Here's how the part is built. I have some questions about the finished solid (model axes, mm). A direction names the side the tool comes from. Round coordinates to 2 decimals unless told otherwise and drop trailing zeros. Write each loop counter-clockwise with the first axis right and the second up, starting at its lowest first coordinate (ties: lowest second). Pieces come first, ordered by that corner, then holes. Notation, with made-up numbers: (-26.75, 70) - (19.25, 70) arc R9 cw to (19.25, 86) - close; hole circle Ø7 at (64, 83). An arc over 180 degrees is marked (long way). One line per question, with ' | ' between items. Start each with the question number.
(1) For faces 4 (the flat face through (-12.5, 0, 5)), 5 (the flat face through (0, 7, 0.5)), 6 (the cylindrical face through (9.6, -4.3, 7.5)), which set-ups out of +Z, -Z, +X, -X, +Y, -Y let a thin tool reach every point of the face, with its end or its side?
(2) Imagine slicing it at B-B (z = 3.25). Write out the boundary of the cut face in (x, y), plus the area to 3 significant figures.
(3) Imagine slicing it at D-D (y = -7). Write out the boundary of the cut face in (x, z), plus the area to 3 significant figures.
(4) Thinking about a two-plate mould opening in X: for faces 1 (the cylindrical face through (-6.98, -11.39, 7.54)), 2 (the cylindrical face through (0.175, 5.452, 6.419)), 3 (the flat face through (-12, -12, 5)), which applies, pulls with the +X half, pulls with the -X half, needs draft (parallel to the pull), parting line crosses it, or undercut?
(5) Imagine slicing it at C-C (x = 6). Write out the boundary of the cut face in (y, z).
(6) If I drill on L1, parallel to Y at x = -6, z = 7.75; L2, parallel to X at y = -10, z = 8.25; L3, parallel to Y at x = 6, z = 6.15, over which ranges is the centre line in solid material (lowest first)?
(7) Imagine slicing it at A-A (y = 7). Write out the boundary of the cut face in (x, z), plus the area to 4 significant figures.
(8) Will this pin go through, and if not, where does the flat tip stop? pin 1 (5.5 mm diameter, centred on x = 6, y = -7, fed in from +Z).
from build123d import *

# Parameters (mm, degrees)
SKETCH1_W           = 25
SKETCH1_H           = 25
BOSS_EXTRUDE1_DEPTH = 10
SKETCH3_R           = 4.5
CUT_EXTRUDE2_DEPTH  = 5
SKETCH4_R           = 2.25
CUT_EXTRUDE3_DEPTH  = 14
SKETCH5_R           = 0.905939467
CUT_EXTRUDE4_DEPTH  = 31
M5_TAPPED_HOLE1_D   = 4.2
CHAMFER1_SIZE       = 1
SKETCH8_W           = 0.5
SKETCH8_H           = 8
CUT_EXTRUDE5_DEPTH  = 31
CHAMFER2_SIZE       = 2


with BuildPart() as part:
    # Sketch1 → Boss-Extrude1 (new body)
    with BuildSketch(Plane.XY):
        Rectangle(SKETCH1_W, SKETCH1_H)
    extrude(amount=BOSS_EXTRUDE1_DEPTH)

    # Sketch3 → Cut-Extrude2 (cut)
    with BuildSketch(Plane.XY.offset(10)):
        with Locations((-6, -7)):
            Circle(SKETCH3_R)
        with Locations(Location((6, -7, 0), (0, 0, 180))):
            Circle(SKETCH3_R)
    extrude(amount=-CUT_EXTRUDE2_DEPTH, mode=Mode.SUBTRACT)

    # Sketch4 → Cut-Extrude3 (cut)
    with BuildSketch(Plane.XY.offset(10)):
        with Locations((-6, -7)):
            Circle(SKETCH4_R)
        with Locations((6, -7)):
            Circle(SKETCH4_R)
    extrude(amount=-CUT_EXTRUDE3_DEPTH, mode=Mode.SUBTRACT)

    # Sketch5 → Cut-Extrude4 (cut)
    with BuildSketch(Plane.ZY.offset(12.5)):
        with Locations(Location((5, 7, 0), (0, 0, 270))):
            Circle(SKETCH5_R)
    extrude(amount=-CUT_EXTRUDE4_DEPTH, mode=Mode.SUBTRACT)

    # M5 Tapped Hole1 (through all)
    with Locations(Plane(origin=(-12.5, 7, 5), x_dir=(0, -1, 0), z_dir=(-1, 0, 0))):
        with Locations((0, 0)):
            Hole(M5_TAPPED_HOLE1_D / 2)

    # Chamfer1
    chamfer1_edges = [part.edges().sort_by_distance(p)[0] for p in [
        (12.5, -12.5, 5),
        (-12.5, -12.5, 5),
        (-12.5, 12.5, 5),
        (12.5, 12.5, 5),
    ]]
    chamfer(chamfer1_edges, length=CHAMFER1_SIZE)

    # Sketch8 → Cut-Extrude5 (cut)
    with BuildSketch(Plane.ZY.offset(12.5)):
        with Locations((0.25, 8.5)):
            Rectangle(SKETCH8_W, SKETCH8_H)
    extrude(amount=-CUT_EXTRUDE5_DEPTH, mode=Mode.SUBTRACT)

    # Chamfer2
    chamfer2_edges = [part.edges().sort_by_distance(p)[0] for p in [
        (0, 12.5, 0.5),
    ]]
    chamfer(chamfer2_edges, length=CHAMFER2_SIZE)


solid = part.part
Check sheet entries:
1) face 4: +Z, -Z, -X, +Y, -Y | face 5: -Z, +X, -X, +Y | face 6: +Z
2) outline: (-12.5, -11.5) - (-11.5, -12.5) - (11.5, -12.5) - (12.5, -11.5) - (12.5, 5.84) - (-12.5, 5.84) - close; (-12.5, 8.16) - (12.5, 8.16) - (12.5, 11.5) - (11.5, 12.5) - (-11.5, 12.5) - (-12.5, 11.5) - close; hole circle Ø4.5 at (-6, -7); hole circle Ø4.5 at (6, -7) | area: 533 mm^2
3) outline: (-12.5, 0) - (-8.25, 0) - (-8.25, 5) - (-10.5, 5) - (-10.5, 10) - (-12.5, 10) - close; (-3.75, 0) - (3.75, 0) - (3.75, 5) - (1.5, 5) - (1.5, 10) - (-1.5, 10) - (-1.5, 5) - (-3.75, 5) - close; (8.25, 0) - (12.5, 0) - (12.5, 10) - (10.5, 10) - (10.5, 5) - (8.25, 5) - close | area: 115 mm^2
4) face 1: undercut | face 2: needs draft | face 3: pulls with the -X half
5) outline: (-12.5, 0) - (-9.25, 0) - (-9.25, 5) - (-11.5, 5) - (-11.5, 10) - (-12.5, 10) - close; (-4.75, 0) - (4.5, 0) - (4.5, 0.5) - (10.5, 0.5) - (12.5, 2.5) - (12.5, 10) - (-2.5, 10) - (-2.5, 5) - (-4.75, 5) - close; hole circle Ø4.2 at (7, 5)
6) L1: -12.5 to -11.5, -2.5 to 12.5 | L2: -12.5 to -9.35, -2.65 to 2.65, 9.35 to 12.5 | L3: -12.5 to -11.5, -2.5 to 5.24, 8.76 to 12.5
7) outline: (-12.5, 0.5) - (12.5, 0.5) - (12.5, 2.9) - (-12.5, 2.9) - close; (-12.5, 7.1) - (12.5, 7.1) - (12.5, 10) - (-12.5, 10) - close | area: 132.5 mm^2
8) pin 1: z = 5
